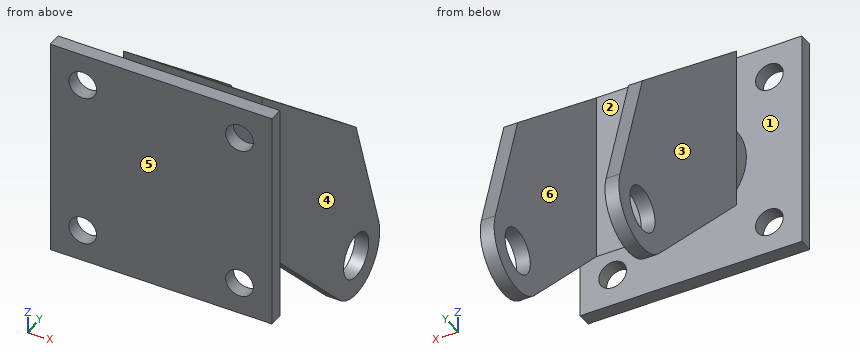
from build123d import *

# Parameters (mm, degrees)
SKETCH1_W                = 80
SKETCH1_H                = 80
SKETCH1_R                = 5
BOSS_EXTRUDE3_DEPTH      = 5
SKETCH3_R                = 20
BOSS_EXTRUDE4_DEPTH      = 15
BOSS_EXTRUDE6_DEPTH      = 25
BOSS_EXTRUDE6_DEPTH_BACK = 25
SKETCH6_R                = 8
CUT_EXTRUDE1_DEPTH       = 50
CUT_EXTRUDE1_DEPTH_BACK  = 25
SKETCH8_W                = 40
SKETCH8_H                = 200


with BuildPart() as part:
    # Sketch1 → Boss-Extrude3 (new body)
    with BuildSketch(Plane(origin=(0, 0, 0), x_dir=(1, 0, 0), z_dir=(0, 1, 0))):
        Rectangle(SKETCH1_W, SKETCH1_H)
        with Locations(Location((-28.284271247, -28.284271247, 0), (0, 0, 270))):
            Circle(SKETCH1_R, mode=Mode.SUBTRACT)
        with Locations(Location((-28.284271247, 28.284271247, 0), (0, 0, 270))):
            Circle(SKETCH1_R, mode=Mode.SUBTRACT)
        with Locations(Location((28.284271247, 28.284271247, 0), (0, 0, 270))):
            Circle(SKETCH1_R, mode=Mode.SUBTRACT)
        with Locations(Location((28.284271247, -28.284271247, 0), (0, 0, 270))):
            Circle(SKETCH1_R, mode=Mode.SUBTRACT)
    extrude(amount=BOSS_EXTRUDE3_DEPTH)

    # Sketch3 → Boss-Extrude4 (add)
    with BuildSketch(Plane(origin=(0, 5, 0), x_dir=(1, 0, 0), z_dir=(0, 1, 0))):
        with Locations(Location((0, 0, 0), (0, 0, 270))):
            Circle(SKETCH3_R)
    extrude(amount=BOSS_EXTRUDE4_DEPTH)

    # Sketch6 → Boss-Extrude6 (add, two sides: drawn at the far end of the back side and taken through both)
    with BuildSketch(Plane(origin=(0, 0, 0), x_dir=(0, 0, -1), z_dir=(1, 0, 0)).offset(-BOSS_EXTRUDE6_DEPTH_BACK)):
        with BuildLine():
            Line((0, 20), (30, 20))
            Line((30, 20), (80.476983059, 69.265344627))
            ThreePointArc((80.476983059, 69.265344627), (82.87355244, 87.698808192), (65.5, 94.309088021))
            Line((65.5, 94.309088021), (20, 80))
            Line((20, 80), (-30, 20))
            Line((-30, 20), (0, 20))
        make_face()
        with Locations((70, 80)):
            Circle(SKETCH6_R, mode=Mode.SUBTRACT)
    extrude(amount=BOSS_EXTRUDE6_DEPTH + BOSS_EXTRUDE6_DEPTH_BACK)

    # Sketch8 → Cut-Extrude1 (cut, two sides: drawn at the far end of the back side and taken through both)
    with BuildSketch(Plane(origin=(0, 80, 0), x_dir=(-1, 0, 0), z_dir=(0, -1, 0)).offset(-CUT_EXTRUDE1_DEPTH_BACK)):
        Rectangle(SKETCH8_W, SKETCH8_H)
    extrude(amount=CUT_EXTRUDE1_DEPTH + CUT_EXTRUDE1_DEPTH_BACK, mode=Mode.SUBTRACT)


solid = part.part
Work out the finished part from the listing and answer in its coordinate system (mm). Face numbers are marked on the shaded views. A direction names the side the tool comes from. Round coordinates to 2 decimals unless told otherwise and drop trailing zeros. Loops run counter-clockwise (first coordinate to the right, second up) from the corner with the lowest first, then second, coordinate; pieces in that order, holes last. Notation, with made-up numbers: (68, 71.5) -> (82, 71.5) arc R26 ccw to (82, 99.5) -> close; hole circle Ø4 at (12.5, -27.5). An arc over 180 degrees is marked (long way). Use one line per item in the form item = value.
(1) Straight lines are drawn through the part: line 1 (X direction, y = 36, z = 5.5); line 2 (Y direction, x = 27, z = -33.5); line 3 (X direction, y = 25.5, z = -20.5). For each, find the intervals that lie inside material, in ascending order.
Answer list:
line_1 = -25 to -20, 20 to 25
line_2 = 0 to 5
line_3 = -25 to 25
(2) Find section A-A on y = 46. Give the vertices of the cut face in (x, z), then the cut area to 3 significant figures.
Answer list:
outline = (-25, -56.64) -> (-20, -56.64) -> (-20, 8.33) -> (-25, 8.33) -> close; (20, -56.64) -> (25, -56.64) -> (25, 8.33) -> (20, 8.33) -> close
area = 650 mm2
(3) Find section C-C on x = 0. Give the vertices of the cut face in (y, z).
Answer list:
outline = (0, -40) -> (5, -40) -> (5, -20) -> (20, -20) -> (20, -30) -> (30, -40.25) -> (30, 21.67) -> (20, 30) -> (20, 20) -> (5, 20) -> (5, 40) -> (0, 40) -> close
(4) For a pull along X with two mould halves and no side action, classify the marked faces 4, 5 and 6 as released by +X, released by -X, zero draft, split by the parting line, or undercut.
Answer list:
face_4 = released by +X
face_5 = zero draft
face_6 = undercut
(5) Flat-ended cylindrical pins translate along their axes: P1, Ø12, axis at x = 20.5, z = -19.5, coming from the +Y side; P2, Ø20, axis at x = -1, z = -23, coming from the +Y side; P3, Ø2.5, axis at x = -6.5, y = 2.5, coming from the -Z side. Find the tip coordinate at first contact, or state that the pin passes through.
Answer list:
P1 = 81.73
P2 = 30
P3 = -40
(6) A tool of negligible diameter and unlimited length cuts with its end or side. For the marked faces 1, 2 and 3, from which of +Z, -Z, +X, -X, +Y, -Y can it reach the whole face along a straight path? Write none if from no direction.
Answer list:
face_1 = none
face_2 = +Z, -Z, +Y
face_3 = +Z, -Z, -X, +Y
(7) Find section D-D on z = -51. Give the vertices of the cut face in (x, y), then the cut area to 3 significant figures.
Answer list:
outline = (-25, 40.5) -> (-20, 40.5) -> (-20, 89.75) -> (-25, 89.75) -> close; (20, 40.5) -> (25, 40.5) -> (25, 89.75) -> (20, 89.75) -> close
area = 493 mm2
(8) Find section B-B on z = 0. Give the vertices of the cut face in (x, y).
Answer list:
outline = (-40, 0) -> (40, 0) -> (40, 5) -> (20, 5) -> (20, 20) -> (25, 20) -> (25, 56) -> (20, 56) -> (20, 30) -> (-20, 30) -> (-20, 56) -> (-25, 56) -> (-25, 20) -> (-20, 20) -> (-20, 5) -> (-40, 5) -> close
